Build history of the part. All positions in model axes, mm. Face numbers are marked on the shaded views. A direction names the side the tool comes from. Give positions to 0.01 mm unless a question says otherwise; leave off trailing zeros. Order: outer loops, then holes, each group sorted by start corner. A loop starts at its lowest first (then second) coordinate and runs counter-clockwise, first axis right, second up. Notation, with made-up numbers: (-28.75, 50.5) - (2.25, 50.5) arc R18 ccw to (2.25, 82.5) - close; hole circle Ø9 at (-33, -12.75). An arc over 180 degrees is marked (long way). Write each question's results on one line, items separated by ' | '. Start each with the question number.
1) Cut at D-D on z = 4.2. List the corners of the cut face in (x, y).
2) Drop flat-ended pins along their axis: pin 1 Ø0.6 at (x, z) = (-1, 3) entering from +Y; pin 2 Ø1.8 at (y, z) = (-5.5, 3.5) entering from +X; pin 3 Ø1 at (y, z) = (5.5, 3.5) entering from -X. Give the stop position or say it passes through.
3) Cut at C-C on z = 3.5. State how many separate pieces and enclosed holes the cut face has, plus the area to 3 significant figures.
4) Cut at A-A on y = -5. List the corners of the cut face in (x, z).
5) Tool access for the marked faces 3, 4 and 5: list every direction of +Z, -Z, +X, -X, +Y, -Y with a clear straight run to the whole face (end or side of a thin tool).
6) Two-plate mould, pull along Y, no slides. Class the marked faces 1 and 2: +Y half, -Y half, draft (parallel to the pull), parting line (faces both ways), or undercut.
7) Drill centre lines: line 1 along Y through (x, z) = (-1.5, 0.3); line 2 along Y through (x, z) = (-0.75, 3.5); line 3 along X through (y, z) = (-6, 1.95). Where is each one in solid material? Low to high. Write a range as from..to.
8) Cut at B-B on x = -1.5. List the corners of the cut face in (y, z), plus the area to 3 significant figures.
from build123d import *

# Parameters (mm, degrees)
SKETCH1_W           = 4
SKETCH1_H           = 16
BOSS_EXTRUDE1_DEPTH = 1
SKETCH2_W           = 0.5
SKETCH2_H           = 15
BOSS_EXTRUDE2_DEPTH = 3.5
SKETCH3_R           = 0.5
CUT_EXTRUDE1_DEPTH  = 4.5
SKETCH4_R           = 0.2
CUT_EXTRUDE2_DEPTH  = 4.5
SKETCH5_W           = 8.19252636
SKETCH5_H           = 8
CUT_EXTRUDE3_DEPTH  = 3.5


with BuildPart() as part:
    # Sketch1 → Boss-Extrude1 (new body)
    with BuildSketch(Plane.XY):
        Rectangle(SKETCH1_W, SKETCH1_H)
    extrude(amount=BOSS_EXTRUDE1_DEPTH)

    # Sketch2 → Boss-Extrude2 (add)
    with BuildSketch(Plane.XY.offset(1)):
        with Locations((0.75, 0)):
            Rectangle(SKETCH2_W, SKETCH2_H)
        with Locations((-0.75, 0)):
            Rectangle(SKETCH2_W, SKETCH2_H)
    extrude(amount=BOSS_EXTRUDE2_DEPTH)

    # Sketch3 → Cut-Extrude1 (cut)
    with BuildSketch(Plane.ZY.offset(1)):
        with Locations((3.5, 5)):
            Circle(SKETCH3_R)
        with Locations((3.5, -5)):
            Circle(SKETCH3_R)
    extrude(amount=-CUT_EXTRUDE1_DEPTH, mode=Mode.SUBTRACT)

    # Sketch4 → Cut-Extrude2 (cut)
    with BuildSketch(Plane.XY.offset(1)):
        with Locations((-1.5, 7.5)):
            Circle(SKETCH4_R)
        with Locations((-1.5, -7.5)):
            Circle(SKETCH4_R)
        with Locations((1.5, -7.5)):
            Circle(SKETCH4_R)
        with Locations((1.5, 7.5)):
            Circle(SKETCH4_R)
    extrude(amount=-CUT_EXTRUDE2_DEPTH, mode=Mode.SUBTRACT)

    # Sketch5 → Cut-Extrude3 (cut)
    with BuildSketch(Plane.XY.offset(4.5)):
        Rectangle(SKETCH5_W, SKETCH5_H)
    extrude(amount=-CUT_EXTRUDE3_DEPTH, mode=Mode.SUBTRACT)


solid = part.part
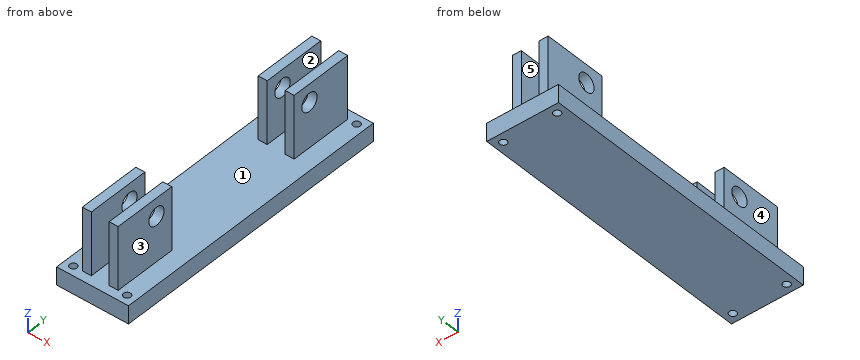
Results:
1) outline: (-1, -7.5) - (-0.5, -7.5) - (-0.5, -4) - (-1, -4) - close; (-1, 4) - (-0.5, 4) - (-0.5, 7.5) - (-1, 7.5) - close; (0.5, -7.5) - (1, -7.5) - (1, -4) - (0.5, -4) - close; (0.5, 4) - (1, 4) - (1, 7.5) - (0.5, 7.5) - close
2) pin 1: y = 7.5 | pin 2: x = 1 | pin 3: x = -1
3) separate pieces: 8 | enclosed holes: 0 | area: 5.00 mm^2
4) outline: (-2, 0) - (2, 0) - (2, 1) - (1, 1) - (1, 3) - (0.5, 3) - (0.5, 1) - (-0.5, 1) - (-0.5, 3) - (-1, 3) - (-1, 1) - (-2, 1) - close; (-1, 4) - (-0.5, 4) - (-0.5, 4.5) - (-1, 4.5) - close; (0.5, 4) - (1, 4) - (1, 4.5) - (0.5, 4.5) - close
5) face 3: +Z, +X, +Y, -Y | face 4: +Z, -X, +Y, -Y | face 5: +Z, +Y, -Y
6) face 1: undercut | face 2: draft
7) line 1: -8..-7.7, -7.3..7.3, 7.7..8 | line 2: -7.5..-5.5, -4.5..-4, 4..4.5, 5.5..7.5 | line 3: -1..-0.5, 0.5..1
8) outline: (-8, 0) - (-7.7, 0) - (-7.7, 1) - (-8, 1) - close; (-7.3, 0) - (7.3, 0) - (7.3, 1) - (-7.3, 1) - close; (7.7, 0) - (8, 0) - (8, 1) - (7.7, 1) - close | area: 15.2 mm^2
